Source: three-view drawing plus pictorial views. Frame: mm from the lowest corner of the part. A direction names the side the tool comes from. Give positions to 0.01 mm unless a question says otherwise; leave off trailing zeros. Order: outer loops, then holes, each group sorted by start corner. A loop starts at its lowest first (then second) coordinate and runs counter-clockwise, first axis right, second up. Notation, with made-up numbers: (38.5, -6) -> (65.5, -6) arc R12 cw to (65.5, 17) -> close; hole circle Ø8 at (67.5, -8.75). An arc over 180 degrees is marked (long way). Write item = value, one per line.
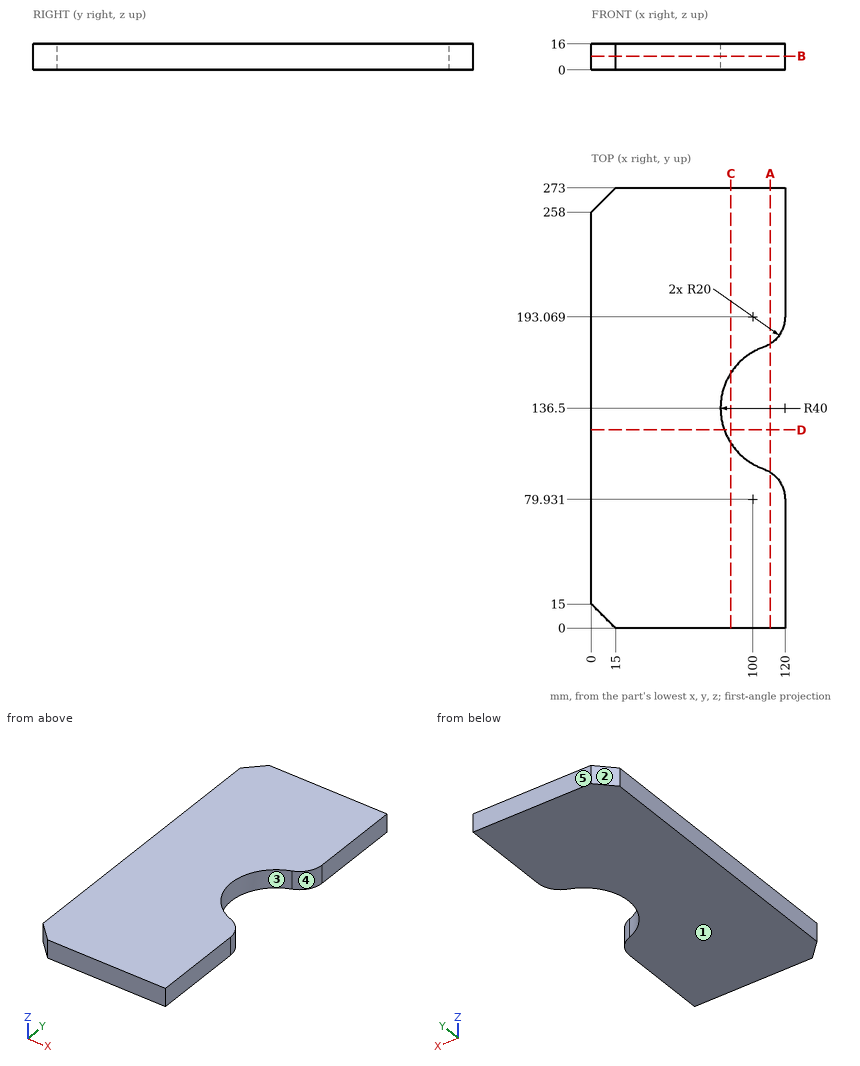
1) Section query D-D (y = 123). Output: boundary loops of the cut face in (x, z), plus the area to 3 significant figures.
Check sheet entries:
outline = (0, 0) -> (82.35, 0) -> (82.35, 16) -> (0, 16) -> close
area = 1,320 mm²
2) Section query B-B (z = 8.5). Output: boundary loops of the cut face in (x, y), plus the area to 3 significant figures.
Check sheet entries:
outline = (0, 15) -> (15, 0) -> (120, 0) -> (120, 79.93) arc R20 ccw to (106.67, 98.79) arc R40 cw to (106.67, 174.21) arc R20 ccw to (120, 193.07) -> (120, 273) -> (15, 273) -> (0, 258) -> close
area = 29,900 mm²
3) Mould query, pull axis Y, two halves, no side actions, for the marked faces 1, 2 and 3. Classes: +Y half, -Y half, draft (parallel to the pull), parting line (faces both ways), or undercut.
Check sheet entries:
face_1 = draft
face_2 = +Y half
face_3 = undercut
4) Reachability of the marked faces 4 and 5 from +Z, -Z, +X, -X, +Y, -Y: full face, straight path, thin tool, end or side. Return the list, or none.
Check sheet entries:
face_4 = +Z, -Z, +X
face_5 = +Z, -Z, +X, -X, +Y
5) Section query A-A (x = 111). Output: boundary loops of the cut face in (y, z) (1 decimal), plus the area to 3 significant figures.
Check sheet entries:
outline = (0, 0) -> (96.6, 0) -> (96.6, 16) -> (0, 16) -> close; (176.4, 0) -> (273, 0) -> (273, 16) -> (176.4, 16) -> close
area = 3,090 mm²
6) First-contact query: P1, Ø8, axis at y = 130, z = 11, coming from the +X side. Flat tip, straight axial feed; report the tip coordinate or a pass-through.
Check sheet entries:
P1 = 81.4
7) Line query: line 1 (Y direction, x = 96.5, z = 1); line 2 (Y direction, x = 111, z = 15) (1 decimal); line 3 (X direction, y = 166.5, z = 15.25) (1 decimal). Output: solid intervals per line, ascending. Write a range as from..to.
Check sheet entries:
line_1 = 0..104.13, 168.87..273
line_2 = 0..96.6, 176.4..273
line_3 = 0..93.5
8) Section query C-C (x = 86.5). Output: boundary loops of the cut face in (y, z), plus the area to 3 significant figures.
Check sheet entries:
outline = (0, 0) -> (114.64, 0) -> (114.64, 16) -> (0, 16) -> close; (158.36, 0) -> (273, 0) -> (273, 16) -> (158.36, 16) -> close
area = 3,670 mm²
